```python
from build123d import *

# Parameters (mm, degrees)
SKETCH_1_R      = 12.5
EXTRUDE_1_DEPTH = 45
SKETCH_2_R      = 25
EXTRUDE_2_DEPTH = 8
SKETCH_3_R      = 10
EXTRUDE_3_DEPTH = 40
SKETCH_5_W      = 2
SKETCH_5_H      = 6
SKETCH_6_R      = 7.5
EXTRUDE_4_DEPTH = 18


with BuildPart() as part:
    # 草图1 → 凸台-拉伸1 (new body)
    with BuildSketch(Plane.XY):
        with Locations(Location((0, 0, 0), (0, 0, 180))):
            Circle(SKETCH_1_R)
    extrude(amount=EXTRUDE_1_DEPTH)

    # 草图2 → 凸台-拉伸2 (add)
    with BuildSketch(Plane(origin=(0, 0, 0), x_dir=(-1, 0, 0), z_dir=(0, 0, -1))):
        Circle(SKETCH_2_R)
    extrude(amount=EXTRUDE_2_DEPTH)

    # 草图3 → 凸台-拉伸3 (add)
    with BuildSketch(Plane.XY.offset(45)):
        Circle(SKETCH_3_R)
    extrude(amount=EXTRUDE_3_DEPTH)

    # 草图5 → 切除-旋转1 (revolve, cut)
    with BuildSketch(Plane(origin=(0, 0, 0), x_dir=(1, 0, 0), z_dir=(0, 1, 0)), mode=Mode.PRIVATE) as cut_revolve_1_sk:
        with Locations((11.5, -3)):
            Rectangle(SKETCH_5_W, SKETCH_5_H)
    revolve(cut_revolve_1_sk.sketch.rotate(Axis((0, 0, 0), (0, 0, 1)), 180), axis=Axis((0, 0, 0), (0, 0, 1)), mode=Mode.SUBTRACT)

    # 草图6 → 凸台-拉伸4 (add)
    with BuildSketch(Plane.XY.offset(85)):
        Circle(SKETCH_6_R)
    extrude(amount=EXTRUDE_4_DEPTH)


solid = part.part
```
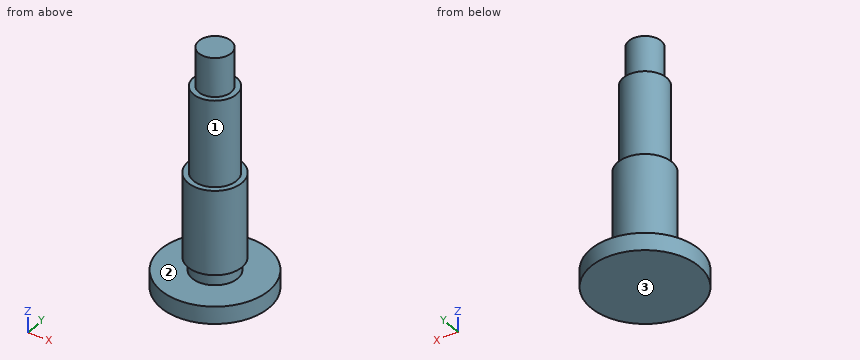
Geometry: final body of the model. Coordinates: model frame, mm. Face numbers are marked on the shaded views. A direction names the side the tool comes from. Round coordinates to 2 decimals unless told otherwise and drop trailing zeros. Write each loop counter-clockwise with the first axis right and the second up, starting at its lowest first coordinate (ties: lowest second). Pieces come first, ordered by that corner, then holes. Notation, with made-up numbers: M 9.25,45.25 L 55.25,45.25 A30 cw 55.25,71.25 Z; hole C -20.75,-28 d2. An arc over 180 degrees is marked long. Answer in a Markdown table with one row per item. Add a question column.
(1) Contact query for flat-ended pins moving along their axis: pin 1 (12 mm diameter, centred on y = -15.5, z = 36, fed in from +X); pin 2 (10 mm diameter, centred on x = 4.5, y = -16.5, fed in from +Z); pin 3 (12 mm diameter, centred on y = 19.5, z = 4, fed in from -X). Output: stop coordinate, or through.
(2) Reachability of the marked faces 1, 2 and 3 from +Z, -Z, +X, -X, +Y, -Y: full face, straight path, thin tool, end or side. Return the list, or none.
(3) Cut plane D-D, the plane y = 22.5. Return the cut outline in (x, z), then the cut area to 3 significant figures.
(4) Ray query, L1, parallel to Z at x = -10, y = -22.5; L2, parallel to Z at x = -7, y = 7.5; L3, parallel to X at y = 2, z = 50.5. Return the intervals inside material, ascending.
(5) Cut plane A-A, the plane x = 0. Return the cut outline in (y, z).
(6) Cut plane C-C, the plane z = 41.5. Return the cut outline in (x, y), then the cut area to 3 significant figures.
Established:
| question | item | result |
|---|---|---|
| 1 | pin 1 | x = 8.12 |
| 1 | pin 2 | z = 45 |
| 1 | pin 3 | x = -19.98 |
| 2 | face 1 | +Z |
| 2 | face 2 | none |
| 2 | face 3 | -Z, +X, -X, +Y, -Y |
| 3 | outline | M -10.9,-8 L 10.9,-8 L 10.9,0 L -10.9,0 Z |
| 3 | area | 174 mm² |
| 4 | L1 | -8 to 0 |
| 4 | L2 | -8 to 45 |
| 4 | L3 | -9.8 to 9.8 |
| 5 | outline | M -25,-8 L 25,-8 L 25,0 L 10.5,0 L 10.5,6 L 12.5,6 L 12.5,45 L 10,45 L 10,85 L 7.5,85 L 7.5,103 L -7.5,103 L -7.5,85 L -10,85 L -10,45 L -12.5,45 L -12.5,6 L -10.5,6 L -10.5,0 L -25,0 Z |
| 6 | outline | C 0,0 d25 |
| 6 | area | 491 mm² |
